Geometry check sheet. Reference: the model listing, model coordinates, mm. Face numbers are marked on the shaded views. A direction names the side the tool comes from. Round coordinates to 2 decimals unless told otherwise and drop trailing zeros. Write each loop counter-clockwise with the first axis right and the second up, starting at its lowest first coordinate (ties: lowest second). Pieces come first, ordered by that corner, then holes. Notation, with made-up numbers: (-11, 28) - (6, 28) arc R19 cw to (6, 64) - close; hole circle Ø6 at (56.5, 78.25). An arc over 180 degrees is marked (long way). Return JSON: item names as keys, results as strings. Group by question number.
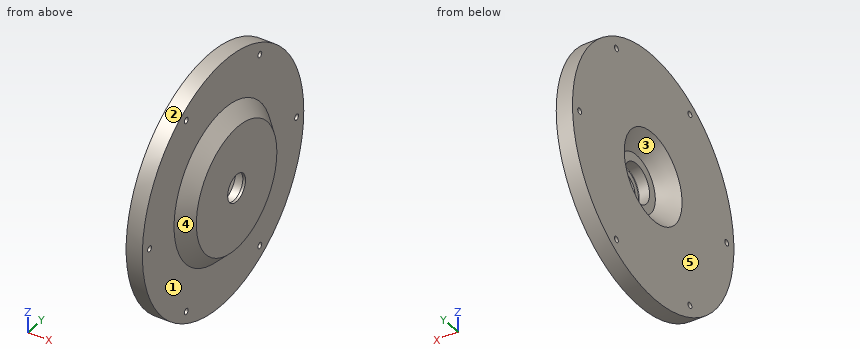
from build123d import *

# Parameters (mm, degrees)
SKETCH2_R          = 5.5
CUT_EXTRUDE1_DEPTH = 85


with BuildPart() as part:
    # Sketch1 → Revolve1 (revolve)
    with BuildSketch(Plane.XY):
        with BuildLine():
            Line((-25, 230.5), (-25, 140))
            Line((-25, 140), (0, 115))
            Line((0, 115), (0, 25.5))
            Line((0, 25.5), (-5, 25.5))
            Line((-5, 25.5), (-5, 35))
            ThreePointArc((-5, 35), (-5.292893219, 35.707106781), (-6, 36))
            Line((-6, 36), (-25, 36))
            Line((-25, 36), (-25, 52.5))
            Line((-25, 52.5), (-55, 82.5))
            Line((-55, 82.5), (-55, 205.5))
            Line((-55, 205.5), (-55, 215.5))
            Line((-55, 215.5), (-55, 230.5))
            Line((-55, 230.5), (-25, 230.5))
        make_face()
    revolve(axis=Axis((5, 0, 0), (-1, 0, 0)))

    # Sketch2 → Cut-Extrude1 (cut)
    with BuildSketch(Plane.ZY.offset(55)):
        with Locations(Location((0, 210, 0), (0, 0, 270))):
            Circle(SKETCH2_R)
        with Locations(Location((181.865334795, 105, 0), (0, 0, 270))):
            Circle(SKETCH2_R)
        with Locations(Location((181.865334795, -105, 0), (0, 0, 270))):
            Circle(SKETCH2_R)
        with Locations(Location((0, -210, 0), (0, 0, 270))):
            Circle(SKETCH2_R)
        with Locations(Location((-181.865334795, -105, 0), (0, 0, 270))):
            Circle(SKETCH2_R)
        with Locations(Location((-181.865334795, 105, 0), (0, 0, 270))):
            Circle(SKETCH2_R)
    extrude(amount=-CUT_EXTRUDE1_DEPTH, mode=Mode.SUBTRACT)


solid = part.part
1. Tool access check on the marked faces 1 and 2. Record the directions out of +Z, -Z, +X, -X, +Y, -Y that give a thin tool (end or side, any length) a straight path to the whole face; none if there is none.
2. Section check A-A (y = 0). Enter the section's corners in (x, z), and give its area (3 significant figures).
3. Section check D-D (x = -48). Enter the section's corners in (y, z).
4. Section check B-B (z = 0). State how many separate pieces and enclosed holes the cut face has, and give its area (3 significant figures).
5. Section check C-C (x = -13). Enter the section's corners in (y, z).
6. Mould release check, pull along Z, two halves, no side actions. Record for the marked faces 3, 4 and 5: pulls with the +Z half, pulls with the -Z half, needs draft (parallel to the pull), parting line crosses it, or undercut.
7. Depth check by flat-ended pin: pin 1 Ø12 at (x, y) = (-47, -134) entering from +Z; pin 2 Ø9 at (y, z) = (-210, 0) entering from -X; pin 3 Ø1 at (x, z) = (-43, 92.5) entering from +Y; pin 4 Ø2 at (y, z) = (-177.5, 120.5) entering from +X. Enter the tip coordinate at first touch or a pass-through.
8. Material ranges on line 1 along Z through (x, y) = (-46, 105); line 2 along X through (y, z) = (33, 144.5); line 3 along Y through (x, z) = (-11, -11.5), recorded low to high.
Result sheet:
{
 "1": {"face 1": "+X", "face 2": "+X, -X"},
 "2": {"outline": "(-55, -230.5) - (-25, -230.5) - (-25, -140) - (0, -115) - (0, -25.5) - (-5, -25.5) - (-5, -35) arc R1 cw to (-6, -36) - (-25, -36) - (-25, -52.5) - (-55, -82.5) - close; (-55, 82.5) - (-25, 52.5) - (-25, 36) - (-6, 36) arc R1 cw to (-5, 35) - (-5, 25.5) - (0, 25.5) - (0, 115) - (-25, 140) - (-25, 230.5) - (-55, 230.5) - close", "area": "14,500 mm²"},
 "3": {"outline": "circle Ø461 at (0, 0); hole circle Ø11 at (-210, 0); hole circle Ø11 at (-105, -181.87); hole circle Ø11 at (-105, 181.87); hole circle Ø151 at (0, 0); hole circle Ø11 at (105, -181.87); hole circle Ø11 at (105, 181.87); hole circle Ø11 at (210, 0)"},
 "4": {"separate pieces": "4", "enclosed holes": "0", "area": "13,800 mm²"},
 "5": {"outline": "circle Ø256 at (0, 0); hole circle Ø72 at (0, 0)"},
 "6": {"face 3": "undercut", "face 4": "parting line crosses it", "face 5": "needs draft"},
 "7": {"pin 1": "stops at z = 191.69", "pin 2": "passes through", "pin 3": "stops at y = 211.34", "pin 4": "stops at x = -25"},
 "8": {"line 1": "z = -205.2 to -187.37, -176.37 to 176.37, 187.37 to 205.2", "line 2": "x = -55 to -25", "line 3": "y = -125.47 to -34.11, 34.11 to 125.47"}
}
